Geometry check sheet. Reference: the model listing, model coordinates, mm. A direction names the side the tool comes from. Round coordinates to 2 decimals unless told otherwise and drop trailing zeros. Write each loop counter-clockwise with the first axis right and the second up, starting at its lowest first coordinate (ties: lowest second). Pieces come first, ordered by that corner, then holes.
Item 1: Draft check along Y on faces 3 (the face through (4, 10, 9)), 4 (the face through (-0.521, 19.966, 12.732)), 5 (the face through (10, 3.2, -2.8)). Enter one of: pulls with the +Y half, pulls with the -Y half, needs draft (parallel to the pull), parting line crosses it, or undercut.
Item 2: Cross-section at A-A (x = 0). Enter the section's corners in (y, z).
Item 3: Access from +Z, -Z, +X, -X, +Y, -Y to the whole of each face (thin tool, end or side, straight path). Record for faces 1 (the face through (20.03, 6.31, 12.04)), 2 (the face through (-0.521, -12.034, 12.732)).
Item 4: Cross-section at D-D (z = -12). Enter the section's corners in (x, y), then the cut area to 3 significant figures.
Item 5: Scan lines: probe 1 along Y at (x, z) = (0, 9.95); probe 2 along Z at (x, y) = (-11.5, -6); probe 3 along Y at (x, z) = (3.5, -7.75). Record each from-to range of solid material in increasing order.
Item 6: Depth check by flat-ended pin: P1, Ø5, axis at x = -16, y = 0, coming from the +Z side; P2, Ø4, axis at y = -15.5, z = 8, coming from the +X side; P3, Ø1.5, axis at y = -3.5, z = 0.5, coming from the -X side. Enter the tip coordinate at first touch or a pass-through.
Item 7: Cross-section at C-C (x = 17). Enter the section's corners in (y, z), then the cut area to 3 significant figures.
from build123d import *

# Parameters (mm, degrees)
SKETCH_1_R                = 10.5
SKETCH_1_R_2              = 6
EXTRUDE_1_DEPTH           = 15
SKETCH_2_R                = 21
SKETCH_2_R_2              = 10.5
EXTRUDE_2_DEPTH           = 6
HOLE_WIZARD_1_D           = 4.5
HOLE_WIZARD_1_DEPTH       = 11.5
HOLE_WIZARD_1_CBORE_D     = 8
HOLE_WIZARD_1_CBORE_DEPTH = 4.6
HOLE_WIZARD_1_TIP         = 1.351936393


with BuildPart() as part:
    # 草图1 → 凸台-拉伸1 (new, symmetric)
    with BuildSketch(Plane.XY):
        Circle(SKETCH_1_R)
        Circle(SKETCH_1_R_2, mode=Mode.SUBTRACT)
    extrude(amount=EXTRUDE_1_DEPTH, both=True)

    # 草图2 → 凸台-拉伸2 (add)
    with BuildSketch(Plane.XY.offset(15)):
        Circle(SKETCH_2_R)
        Circle(SKETCH_2_R_2, mode=Mode.SUBTRACT)
    extrude(amount=-EXTRUDE_2_DEPTH)

    # 打孔尺寸(%根据)内六角圆柱头螺钉的类型1
    with Locations(Plane.XY.offset(15)):
        with Locations((0, 16), (16, 0), (0, -16), (-16, 0)):
            CounterBoreHole(HOLE_WIZARD_1_D / 2, HOLE_WIZARD_1_CBORE_D / 2, HOLE_WIZARD_1_CBORE_DEPTH, depth=HOLE_WIZARD_1_DEPTH)
            with Locations((0, 0, -(HOLE_WIZARD_1_DEPTH + HOLE_WIZARD_1_TIP / 2))):  # 118° drill point
                Cone(0, HOLE_WIZARD_1_D / 2, HOLE_WIZARD_1_TIP, mode=Mode.SUBTRACT)


solid = part.part
Resolved:
1. face 3: needs draft
1. face 4: undercut
1. face 5: parting line crosses it
2. outline: (-21, 9) - (-18.25, 9) - (-18.25, 10.4) - (-20, 10.4) - (-20, 15) - (-21, 15) - close; (-13.75, 9) - (-10.5, 9) - (-10.5, -15) - (-6, -15) - (-6, 15) - (-12, 15) - (-12, 10.4) - (-13.75, 10.4) - close; (6, -15) - (10.5, -15) - (10.5, 9) - (13.75, 9) - (13.75, 10.4) - (12, 10.4) - (12, 15) - (6, 15) - close; (18.25, 9) - (21, 9) - (21, 15) - (20, 15) - (20, 10.4) - (18.25, 10.4) - close
3. face 1: +Z, -Z
3. face 2: +Z
4. outline: circle Ø21 at (0, 0); hole circle Ø12 at (0, 0)
4. area: 233 mm2
5. probe 1: y = -21 to -18.25, -13.75 to -6, 6 to 13.75, 18.25 to 21
5. probe 2: z = 9 to 15
5. probe 3: y = -9.9 to -4.87, 4.87 to 9.9
6. P1: stops at z = 10.4
6. P2: stops at x = 15.86
6. P3: stops at x = -10.13
7. outline: (-12.33, 9) - (-2.02, 9) - (-2.02, 10.4) - (-3.87, 10.4) - (-3.87, 15) - (-12.33, 15) - close; (2.02, 9) - (12.33, 9) - (12.33, 15) - (3.87, 15) - (3.87, 10.4) - (2.02, 10.4) - close
7. area: 107 mm2
